Drawing for the job (mm, zero at the part's lowest x, y, z). A direction names the side the tool comes from. Round coordinates to 2 decimals unless told otherwise and drop trailing zeros. Write each loop counter-clockwise with the first axis right and the second up, starting at its lowest first coordinate (ties: lowest second). Pieces come first, ordered by that corner, then holes. Notation, with made-up numbers: M -14,2 L 13,2 A24 ccw 13,31 Z; hole C 45.5,19.25 d5. An arc over 180 degrees is marked long. Use a Markdown table: item, result. Add a question column.
1) Which spindle directions (+Z, -Z, +X, -X, +Y, -Y) get a long thin tool onto all of the face, cutting with end or side? Do the marked faces 1 and 2. Say none if no direction does.
2) Drop flat-ended pins along their axis: P1, Ø2, axis at y = 11.5, z = 1.5, coming from the -X side; P2, Ø1, axis at x = 31.5, y = 2.5, coming from the -Z side; P3, Ø3, axis at x = 41, y = 10.5, coming from the -Z side; P4, Ø1.5, axis at x = 18.5, z = 4, coming from the -Y side. Give the stop position or say it passes through.
3) Slice it at A-A on x = 29. Write the cut outline in (y, z), plus the area to 3 significant figures.
4) Wall check: probe 1 along Y at (x, z) = (20.5, 6.25); probe 2 along X at (y, z) = (1.5, 8); probe 3 along Y at (x, z) = (32, 8.75) (1 decimal). Give the ranges that are in metal, low to high.
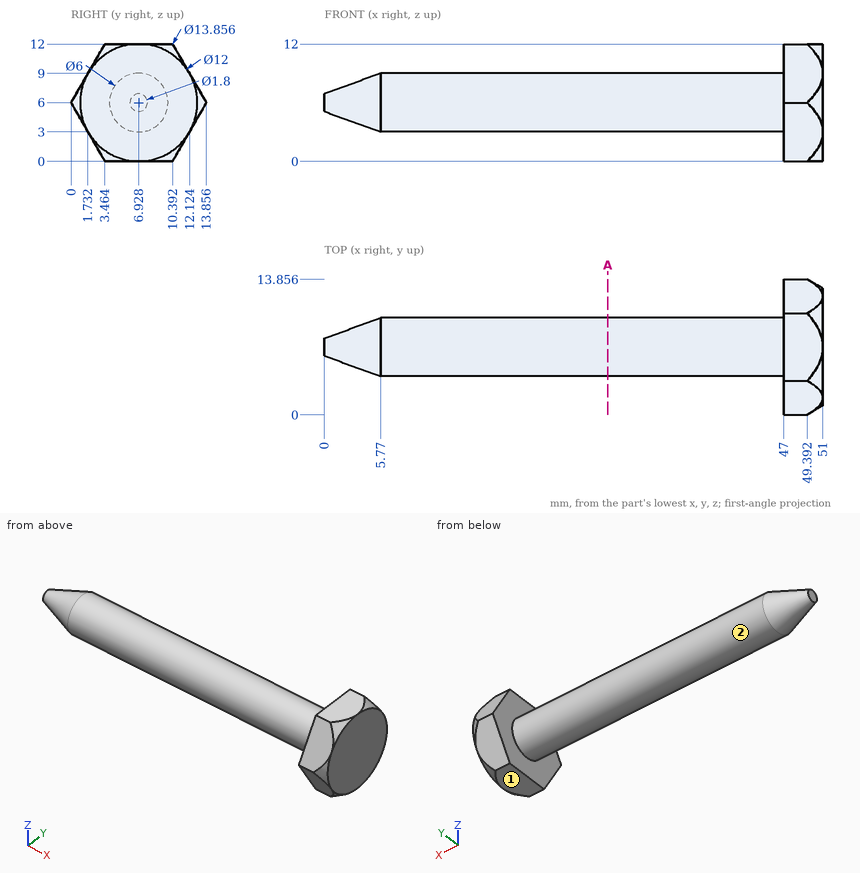
Entries:
| question | item | result |
|---|---|---|
| 1 | face 1 | -Z, +X, -X, +Y, -Y |
| 1 | face 2 | -X |
| 2 | P1 | stops at x = 47 |
| 2 | P2 | passes through |
| 2 | P3 | stops at z = 3.83 |
| 2 | P4 | stops at y = 4.2 |
| 3 | outline | C 6.93,6 d6 |
| 3 | area | 28.3 mm^2 |
| 4 | probe 1 | y = 3.94 to 9.92 |
| 4 | probe 2 | x = 47 to 51 |
| 4 | probe 3 | y = 5.7 to 8.1 |
